```python
from build123d import *

# Parameters (mm, degrees)
BASE_PLATE_DEPTH      = 15
UPRIGHT_WALL_SKETCH_W = 15
UPRIGHT_WALL_SKETCH_H = 50
UPRIGHT_WALL_DEPTH    = 65
WALL_BOSS_SKETCH_R    = 15
WALL_BOSS_DEPTH       = 20
BOSS_BORE_SKETCH_R    = 10
BOSS_BORE_10_DEPTH    = 20
RAISED_BLOCK_SKETCH_W = 15
RAISED_BLOCK_SKETCH_H = 50
RAISED_BLOCK_DEPTH    = 30
LUG_HOLE_SKETCH_R     = 10
LUG_HOLE_DEPTH        = 15


with BuildPart() as part:
    # Base Plate Sketch → Base Plate (new body)
    with BuildSketch(Plane(origin=(0, 0, 0), x_dir=(1, 0, 0), z_dir=(0, 1, 0))):
        with BuildLine():
            Line((-65, -25), (40, -25))
            ThreePointArc((40, -25), (65, 0), (40, 25))
            Line((40, 25), (-65, 25))
            Line((-65, 25), (-65, -25))
        make_face()
    extrude(amount=BASE_PLATE_DEPTH)

    # Upright Wall Sketch → Upright Wall (add)
    with BuildSketch(Plane(origin=(0, 15, 0), x_dir=(1, 0, 0), z_dir=(0, 1, 0))):
        with Locations((-57.5, 0)):
            Rectangle(UPRIGHT_WALL_SKETCH_W, UPRIGHT_WALL_SKETCH_H)
    extrude(amount=UPRIGHT_WALL_DEPTH)

    # Wall Boss Sketch → Wall Boss (add)
    with BuildSketch(Plane(origin=(-50, 0, 0), x_dir=(0, 0, -1), z_dir=(1, 0, 0))):
        with Locations(Location((0, 58, 0), (0, 0, 180))):
            Circle(WALL_BOSS_SKETCH_R)
    extrude(amount=WALL_BOSS_DEPTH)

    # Boss Bore Sketch → Boss Bore Ø10 (cut)
    with BuildSketch(Plane(origin=(-30, 0, 0), x_dir=(0, 0, -1), z_dir=(1, 0, 0))):
        with Locations((0, 58)):
            Circle(BOSS_BORE_SKETCH_R)
    extrude(amount=-BOSS_BORE_10_DEPTH, mode=Mode.SUBTRACT)

    # Raised Block Sketch → Raised Block (add)
    with BuildSketch(Plane(origin=(0, 15, 0), x_dir=(1, 0, 0), z_dir=(0, 1, 0))):
        with Locations((7.5, 0)):
            Rectangle(RAISED_BLOCK_SKETCH_W, RAISED_BLOCK_SKETCH_H)
    extrude(amount=RAISED_BLOCK_DEPTH)

    # Lug Hole Sketch → Lug Hole (cut)
    with BuildSketch(Plane(origin=(0, 15, 0), x_dir=(1, 0, 0), z_dir=(0, 1, 0))):
        with Locations(Location((40, 0, 0), (0, 0, 270))):
            Circle(LUG_HOLE_SKETCH_R)
    extrude(amount=-LUG_HOLE_DEPTH, mode=Mode.SUBTRACT)


solid = part.part
```
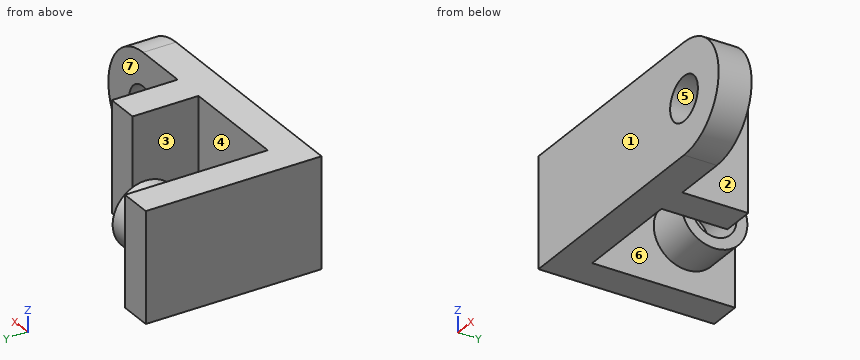
Can you work these out from the model? Positions are in its coordinate system, mm. Face numbers are marked on the shaded views. A direction names the side the tool comes from. Coordinates: 2 decimals unless noted, no trailing zeros. Loops run counter-clockwise (first coordinate to the right, second up) from the corner with the lowest first, then second, coordinate; pieces in that order, holes last. Notation, with made-up numbers: M -16,51.25 L 0,51.25 A17 cw 0,57.25 Z; hole C 87.5,-22.75 d6. An arc over 180 degrees is marked long. Put each result on its own line as item: value. Start each with the question number.
(1) Will these pins go through, and if not, where does the flat tip stop? pin 1 Ø15 at (x, z) = (36.5, 8.5) entering from +Y; pin 2 Ø9 at (y, z) = (24.5, 4.5) entering from +X; pin 3 Ø12 at (x, z) = (8, 10) entering from +Y.
(2) Imagine slicing it at B-B on y = 21. List the corners of the cut face in (x, z) for me.
(3) I need wall thicknesses on probe 1 along Y at (x, z) = (-41, 0); probe 2 along X at (y, z) = (17.5, 16.5); probe 3 along Y at (x, z) = (-47.5, -5). Which ranges of each line are inside material? Lowest first, please.
(4) Which directions (+Z, -Z, +X, -X, +Y, -Y) give clear straight access to the entire face, cutting with the end or side of a thin tool? Please do the marked faces 5, 6 and 7.
(5) Imagine slicing it at D-D on z = -7.5. List the corners of the cut face in (x, y) for me, and give its area (3 significant figures).
(6) We'd pull the mould along X, two halves only. Please class the marked faces 1, 2, 3 and 4: +X half, -X half, draft (parallel to the pull), parting line (faces both ways), or undercut.
(7) Imagine slicing it at A-A on z = 0. List the corners of the cut face in (x, y) for me.
(8) Imagine slicing it at C-C on y = 58. List the corners of the cut face in (x, z) for me, and give its area (3 significant figures).
Worked answers:
1. pin 1: stops at y = 15
1. pin 2: stops at x = 15
1. pin 3: stops at y = 45
2. outline: M -65,-25 L -50,-25 L -50,25 L -65,25 Z; M 0,-25 L 15,-25 L 15,25 L 0,25 Z
3. probe 1: y = 0 to 15, 43 to 48, 68 to 73
3. probe 2: x = -65 to -50, 0 to 15
3. probe 3: y = 0 to 15, 43.86 to 49.34, 66.66 to 72.14
4. face 5: +Y, -Y
4. face 6: none
4. face 7: +Z, -Z, +X, +Y
5. outline: M -65,0 L 33.39,0 L 33.39,15 L 15,15 L 15,45 L 0,45 L 0,15 L -50,15 L -50,45.01 L -30,45.01 L -30,51.39 L -50,51.39 L -50,64.61 L -30,64.61 L -30,70.99 L -50,70.99 L -50,80 L -65,80 Z; M 46.61,0 L 63.85,0 L 63.85,15 L 46.61,15 Z
5. area: 3,410 mm2
6. face 1: draft
6. face 2: +X half
6. face 3: undercut
6. face 4: undercut
7. outline: M -65,0 L 30,0 L 30,15 L 15,15 L 15,45 L 0,45 L 0,15 L -50,15 L -50,43 L -30,43 L -30,48 L -50,48 L -50,68 L -30,68 L -30,73 L -50,73 L -50,80 L -65,80 Z; M 50,0 L 65,0 L 65,15 L 50,15 Z
8. outline: M -65,-25 L -50,-25 L -50,-15 L -30,-15 L -30,-10 L -50,-10 L -50,10 L -30,10 L -30,15 L -50,15 L -50,25 L -65,25 Z
8. area: 950 mm2
